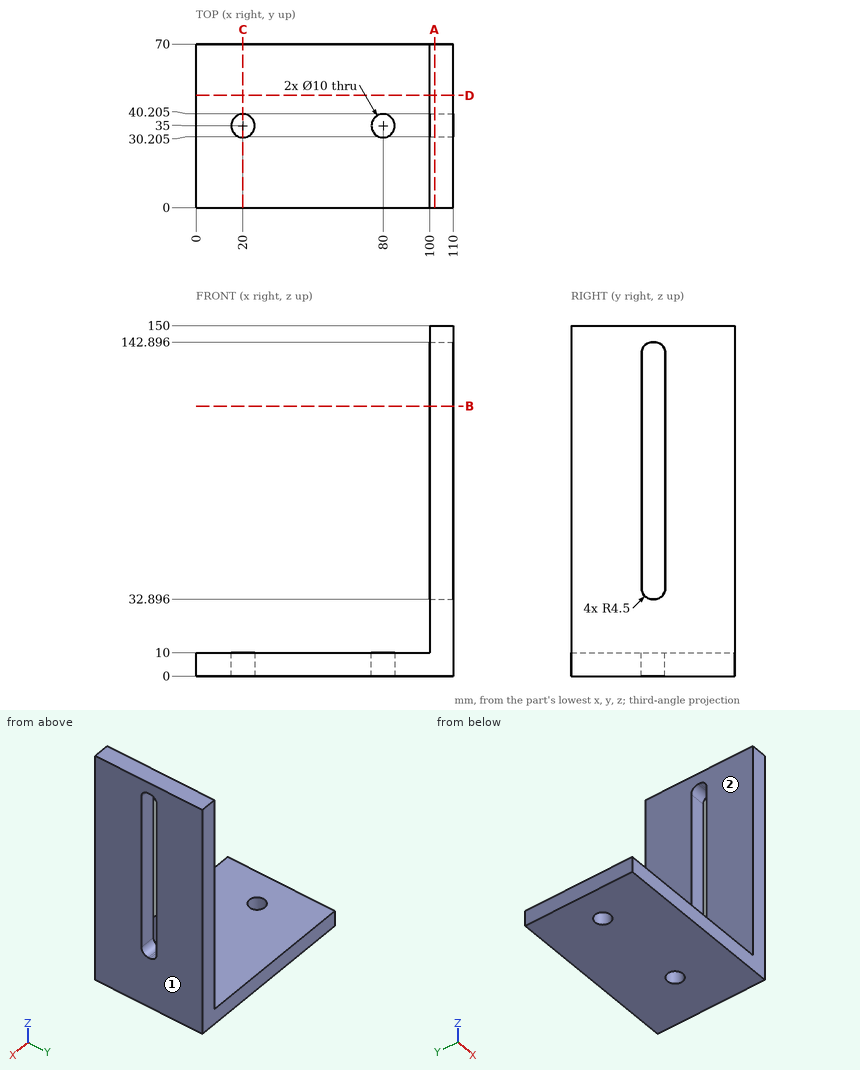
Could you check a few things on this drawing? It's one solid part, dimensions in mm from its lowest x, y, z. A direction names the side the tool comes from. Coordinates: 2 decimals unless noted, no trailing zeros. Order: outer loops, then holes, each group sorted by start corner. A loop starts at its lowest first (then second) coordinate and runs counter-clockwise, first axis right, second up. Notation, with made-up numbers: (76, 47) -> (128, 47) arc R30 ccw to (128, 77) -> close; hole circle Ø4 at (77, 13). An arc over 180 degrees is marked (long way). One line per item, written item: value. Start each with the question number.
1) Imagine slicing it at B-B on z = 115.5. List the corners of the cut face in (x, y) for me (1 decimal).
2) Imagine slicing it at D-D on y = 48. List the corners of the cut face in (x, z) for me, plus the area to 3 significant figures.
3) If I drill on L1, parallel to Y at x = 20, z = 3; L2, parallel to Y at x = 104, z = 37; L3, parallel to X at y = 65.5, z = 95, over which ranges is the centre line in solid material (lowest first)? Write a range as [from, to].
4) Imagine slicing it at C-C on x = 20. List the corners of the cut face in (y, z) for me, plus the area to 3 significant figures.
5) I'm going to push flat-ended pins straight in: pin 1 (12 mm diameter, centred on x = 23, y = 54.5, fed in from +Z); pin 2 (10 mm diameter, centred on y = 27, z = 26, fed in from -X). Where does each tip first touch, or does it pass through?
6) Which directions (+Z, -Z, +X, -X, +Y, -Y) give clear straight access to the entire face, cutting with the end or side of a thin tool? Please do the marked faces 1 and 2.
7) Imagine slicing it at A-A on x = 102. List the corners of the cut face in (y, z) for me (1 decimal), plus the area to 3 significant figures.
Answer list:
1. outline: (100, 0) -> (110, 0) -> (110, 30.2) -> (100, 30.2) -> close; (100, 40.2) -> (110, 40.2) -> (110, 70) -> (100, 70) -> close
2. outline: (0, 0) -> (110, 0) -> (110, 150) -> (100, 150) -> (100, 10) -> (0, 10) -> close
2. area: 2,500 mm2
3. L1: y = [0, 30], [40, 70]
3. L2: y = [0, 30.22], [40.19, 70]
3. L3: x = [100, 110]
4. outline: (0, 0) -> (30, 0) -> (30, 10) -> (0, 10) -> close; (40, 0) -> (70, 0) -> (70, 10) -> (40, 10) -> close
4. area: 600 mm2
5. pin 1: stops at z = 10
5. pin 2: stops at x = 100
6. face 1: +Z, -Z, +X, +Y, -Y
6. face 2: +Z, -X, +Y, -Y
7. outline: (0, 0) -> (70, 0) -> (70, 150) -> (0, 150) -> close; hole (30.2, 37.4) arc R4.5 ccw to (34.7, 32.9) -> (35.7, 32.9) arc R4.5 ccw to (40.2, 37.4) -> (40.2, 138.4) arc R4.5 ccw to (35.7, 142.9) -> (34.7, 142.9) arc R4.5 ccw to (30.2, 138.4) -> close
7. area: 9,420 mm2
